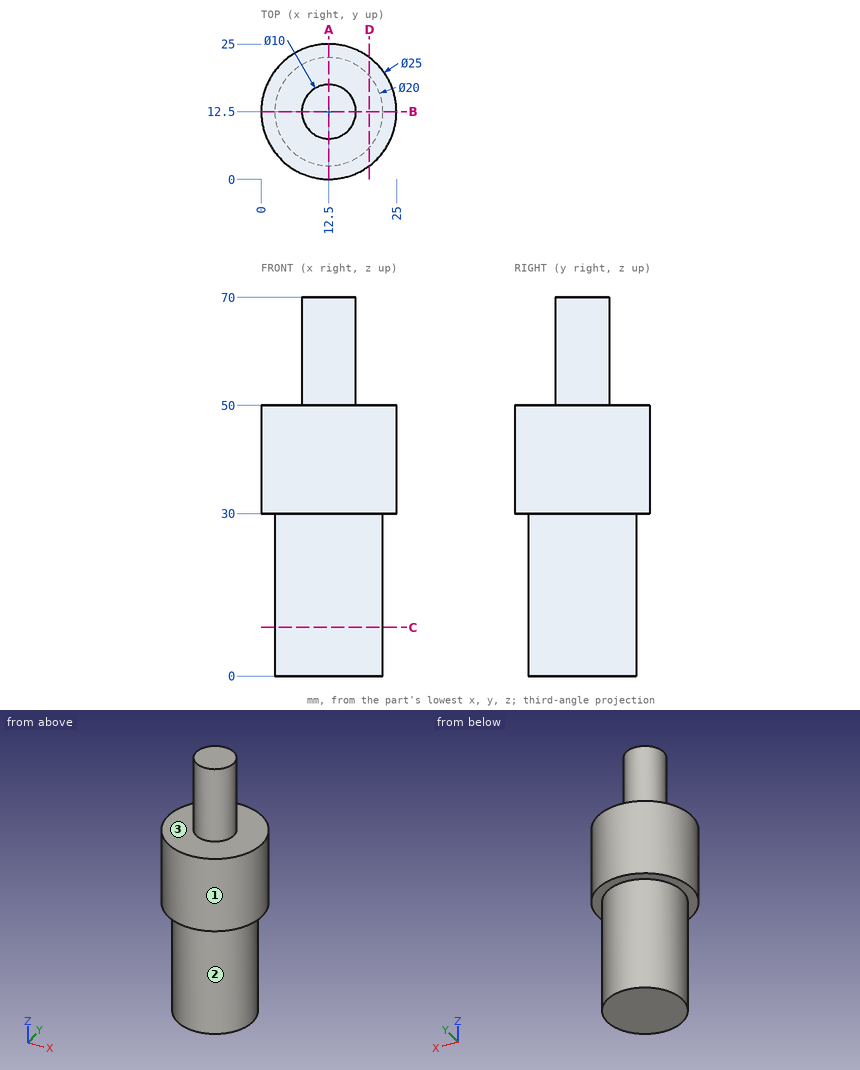
Print and shaded views of the part. All mm, measured from the part's lowest x, y and z. A direction names the side the tool comes from. Coordinates: 2 decimals unless noted, no trailing zeros. Order: outer loops, then holes, each group sorted by start corner. A loop starts at its lowest first (then second) coordinate and runs counter-clockwise, first axis right, second up. Notation, with made-up numbers: M 3,67.25 L 22,67.25 A8 cw 22,80.25 Z; hole C 15.5,26.25 d3. An arc over 180 degrees is marked long. One line per question, with ' | ' between items. Start each with the question number.
Q1. Saw through at D-D (x = 20). List the corners of the cut face in (y, z), then the cut area to 3 significant figures.
Q2. 3-axis set-ups, long thin cutter, end or side, ignore diameter. For the marked faces 1, 2 and 3: which of +Z, -Z, +X, -X, +Y, -Y reach the whole face in a straight line?
Q3. Saw through at C-C (z = 9). List the corners of the cut face in (x, y), then the cut area to 3 significant figures.
Q4. Saw through at A-A (x = 12.5). List the corners of the cut face in (y, z).
Q5. Flat gauge pins, fed straight in: pin 1 Ø1 at (x, z) = (10.5, 32) entering from +Y; pin 2 Ø10 at (y, z) = (4.5, 57) entering from -X; pin 3 Ø4 at (y, z) = (9, 43.5) entering from +X. Where does each tip first touch, or does it go through?
Q6. Probe L1, parallel to Z at x = 22.5, y = 15.75; L2, parallel to Z at x = 18.5, y = 10; L3, parallel to Y at x = 8.25, z = 45. List the from-to ranges inside material, lowest first. Write a range as from..to.
Check values:
1) outline: M 2.5,30 L 5.89,30 L 5.89,0 L 19.11,0 L 19.11,30 L 22.5,30 L 22.5,50 L 2.5,50 Z | area: 797 mm2
2) face 1: +Z, -Z | face 2: -Z | face 3: +Z
3) outline: C 12.5,12.5 d20 | area: 314 mm2
4) outline: M 0,30 L 2.5,30 L 2.5,0 L 22.5,0 L 22.5,30 L 25,30 L 25,50 L 17.5,50 L 17.5,70 L 7.5,70 L 7.5,50 L 0,50 Z
5) pin 1: stops at y = 24.91 | pin 2: stops at x = 8.5 | pin 3: stops at x = 24.91
6) L1: z = 30..50 | L2: z = 0..50 | L3: y = 0.74..24.26
